For this review, take the finished solid that the model builds, in its own axes (mm). Face numbers are marked on the shaded views. Give positions to 0.01 mm unless a question says otherwise; leave off trailing zeros. Write each loop counter-clockwise with the first axis right and the second up, starting at its lowest first coordinate (ties: lowest second). Pieces come first, ordered by that corner, then holes. Notation, with made-up numbers: M 17.25,81 L 44.25,81 A25 cw 44.25,94 Z; hole C 48.5,-11 d5. An arc over 180 degrees is marked long. Use one line per item in the form item = value. Start each with the question number.
Q1. Consider section B-B on x = 100. Write out the cut boundary in (y, z).
Q2. For probe 1 along X at (y, z) = (-0.75, 60); probe 2 along Z at (x, y) = (102, -2); probe 3 along Z at (x, y) = (-95, 3.75) (3 decimals), list the stretches that pass through material, from the lowest coordinate up. Write a range as [from, to].
Q3. Mouldability with a two-part tool opening along Y and no side actions: class the marked faces 1 and 2 as released by +Y, released by -Y, zero draft, split by the parting line, or undercut.
Q4. Consider section A-A on z = 60. Write out the cut boundary in (x, y).
```python
from build123d import *

# Parameters (mm, degrees)
SKETCH1_W      = 310
SKETCH1_H      = 180
SKETCH1_R      = 8
EXTRUDE1_DEPTH = 6


with BuildPart() as part:
    # Sketch1 → Extrude1 (new, symmetric)
    with BuildSketch(Plane(origin=(0, 0, 0), x_dir=(1, 0, 0), z_dir=(0, 1, 0))):
        Rectangle(SKETCH1_W, SKETCH1_H)
        with Locations(Location((100, -60, 0), (0, 0, 270))):
            Circle(SKETCH1_R, mode=Mode.SUBTRACT)
        with Locations(Location((-100, -60, 0), (0, 0, 270))):
            Circle(SKETCH1_R, mode=Mode.SUBTRACT)
        with Locations(Location((-100, 60, 0), (0, 0, 270))):
            Circle(SKETCH1_R, mode=Mode.SUBTRACT)
        with Locations(Location((100, 60, 0), (0, 0, 270))):
            Circle(SKETCH1_R, mode=Mode.SUBTRACT)
    extrude(amount=EXTRUDE1_DEPTH, both=True)


solid = part.part
```
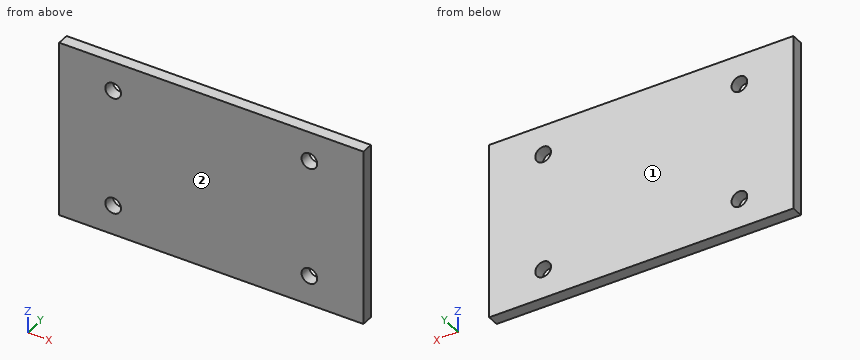
Working result:
q1.outline = M -6,-90 L 6,-90 L 6,-68 L -6,-68 Z; M -6,-52 L 6,-52 L 6,52 L -6,52 Z; M -6,68 L 6,68 L 6,90 L -6,90 Z
q2.probe_1 = [-155, -108], [-92, 92], [108, 155]
q2.probe_2 = [-90, -67.75], [-52.25, 52.25], [67.75, 90]
q2.probe_3 = [-90, -66.245], [-53.755, 53.755], [66.245, 90]
q3.face_1 = released by +Y
q3.face_2 = released by -Y
q4.outline = M -155,-6 L -108,-6 L -108,6 L -155,6 Z; M -92,-6 L 92,-6 L 92,6 L -92,6 Z; M 108,-6 L 155,-6 L 155,6 L 108,6 Z
